from build123d import *

# Parameters (mm, degrees)
SKETCH1_R           = 200
SKETCH1_R_2         = 137.5
SKETCH1_R_3         = 12.5
BOSS_EXTRUDE1_DEPTH = 25
CHAMFER1_SIZE       = 1
SKETCH4_R           = 177.5
CUT_EXTRUDE2_DEPTH  = 5
FILLET1_R           = 2
CHAMFER2_SIZE       = 1


with BuildPart() as part:
    # Sketch1 → Boss-Extrude1 (new body)
    with BuildSketch(Plane.XY):
        Circle(SKETCH1_R)
        Circle(SKETCH1_R_2, mode=Mode.SUBTRACT)
        with Locations((0, 160)):
            Circle(SKETCH1_R_3, mode=Mode.SUBTRACT)
        with Locations((113.13708499, 113.13708499)):
            Circle(SKETCH1_R_3, mode=Mode.SUBTRACT)
        with Locations((160, 0)):
            Circle(SKETCH1_R_3, mode=Mode.SUBTRACT)
        with Locations((113.13708499, -113.13708499)):
            Circle(SKETCH1_R_3, mode=Mode.SUBTRACT)
        with Locations((0, -160)):
            Circle(SKETCH1_R_3, mode=Mode.SUBTRACT)
        with Locations((-113.13708499, -113.13708499)):
            Circle(SKETCH1_R_3, mode=Mode.SUBTRACT)
        with Locations((-160, 0)):
            Circle(SKETCH1_R_3, mode=Mode.SUBTRACT)
        with Locations((-113.13708499, 113.13708499)):
            Circle(SKETCH1_R_3, mode=Mode.SUBTRACT)
    extrude(amount=BOSS_EXTRUDE1_DEPTH)

    # Chamfer1
    chamfer1_edges = [part.edges().sort_by_distance(p)[0] for p in [
        (-200, 0, 0),
        (-200, 0, 25),
        (-137.5, 0, 0),
        (-137.5, 0, 25),
    ]]
    chamfer(chamfer1_edges, length=CHAMFER1_SIZE)

    # Sketch4 → Cut-Extrude2 (cut)
    with BuildSketch(Plane(origin=(0, 0, 0), x_dir=(-1, 0, 0), z_dir=(0, 0, -1))):
        Circle(SKETCH4_R)
    extrude(amount=-CUT_EXTRUDE2_DEPTH, mode=Mode.SUBTRACT)

    # Fillet1
    fillet1_edges = [part.edges().sort_by_distance(p)[0] for p in [
        (177.5, 0, 5),
    ]]
    fillet(fillet1_edges, radius=FILLET1_R)

    # Chamfer2
    chamfer2_edges = [part.edges().sort_by_distance(p)[0] for p in [
        (-137.5, 0, 5),
        (177.5, 0, 0),
    ]]
    chamfer(chamfer2_edges, length=CHAMFER2_SIZE)


solid = part.part
Build history of the part. All positions in model axes, mm. A direction names the side the tool comes from. Coordinates: 2 decimals unless noted, no trailing zeros.
(1) Mould opens along X. For faces 1 (the flat face through (41, 135, 25)), 2 (the cylindrical face through (-125.625, 113.687, 14.86)), 3 (the cylindrical face through (190.764, 60.075, 12.339)) say: pulls with the +X half, pulls with the -X half, needs draft (parallel to the pull), parting line crosses it, or undercut.
(2) 3-axis set-ups, long thin cutter, end or side, ignore diameter. For faces 4 (the flat face through (-51, -129, 5)), 5 (the cylindrical face through (-115.85, -125.34, 14.86)): which of +Z, -Z, +X, -X, +Y, -Y reach the whole face in a straight line?
(3) Drill centre lines: line 1 (X direction, y = 1, z = 20.75); line 2 (Y direction, x = 0, z = 19); line 3 (X direction, y = 11, z = 20.75). Where is each one in solid material? Low to high.
(4) Pin check, flat tips, straight feed: pin 1 Ø12 at (x, y) = (-123, 52) entering from -Z; pin 2 Ø3 at (y, z) = (-22.5, 9) entering from +X; pin 3 Ø1.5 at (y, z) = (-50, 14.5) entering from +X. Stop position of each tip, or through.
(5) Cut at A-A on y = 0. State how many separate pieces and enclosed holes the cut face has, and give its area (3 significant figures).
Working result:
1. face 1: needs draft
1. face 2: undercut
1. face 3: parting line crosses it
2. face 4: -Z
2. face 5: +Z, -Z
3. line 1: x = -200 to -172.46, -147.54 to -137.5, 137.5 to 147.54, 172.46 to 200
3. line 2: y = -200 to -172.5, -147.5 to -137.5, 137.5 to 147.5, 172.5 to 200
3. line 3: x = -199.7 to -165.94, -154.06 to -137.06, 137.06 to 154.06, 165.94 to 199.7
4. pin 1: stops at z = 5
4. pin 2: stops at x = 198.89
4. pin 3: stops at x = 193.84
5. separate pieces: 4
5. enclosed holes: 0
5. area: 1,720 mm2
